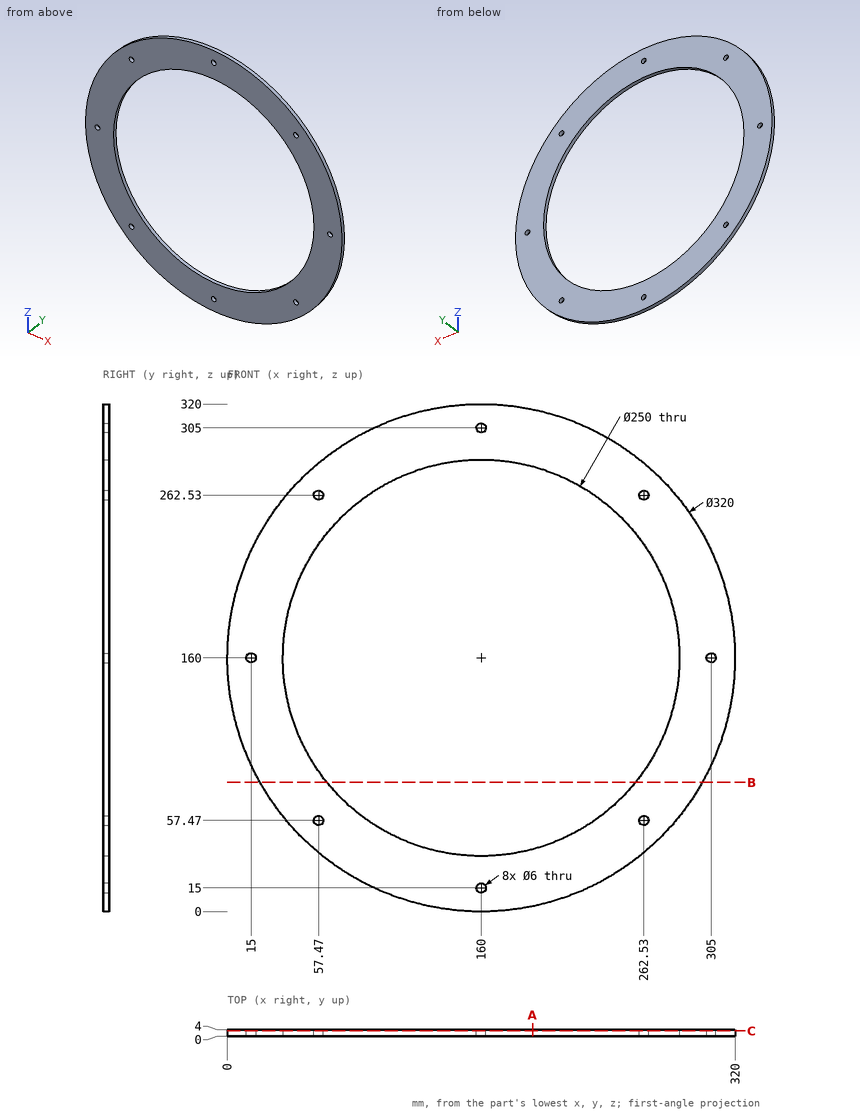
Answer from the drawing. Dimensions are ordinates in mm from the lowest x, y and z of the part. Coordinates: 2 decimals unless noted, no trailing zeros. Write each loop counter-clockwise with the first axis right and the second up, starting at its lowest first coordinate (ties: lowest second). Pieces come first, ordered by that corner, then holes. Notation, with made-up numbers: M -37,77 L -22,77 A6 cw -22,88 Z; hole C 19,-29 d7. An arc over 180 degrees is marked long. Put each result on its own line as item: value. Start each with the question number.
1. Flat-ended cylindrical pins translate along their axes: P1, Ø5.5, axis at x = 57.47, z = 262.53, coming from the -Y side; P2, Ø1, axis at x = 238.5, y = 3, coming from the -Z side; P3, Ø1.5, axis at y = 3, z = 108, coming from the -X side. Find the tip coordinate at first contact, or state that the pin passes through.
2. A cutting plane is placed at B-B on z = 81.5. Write down the section's boundary in (x, y).
3. A cutting plane is placed at A-A on x = 192.5. Write down the section's boundary in (y, z) (1 decimal).
4. A cutting plane is placed at C-C on y = 3.2. Count the separate pieces of the cut face and the enclosed holes in it, then the cut area to 3 significant figures.
5. Consider line 1 (X direction, y = 2.05, z = 55.5) (1 decimal); line 2 (X direction, y = 2.5, z = 179); line 3 (X direction, y = 3.15, z = 15) (1 decimal). Determine where each line is inside the solid, lowest interval first. Write a range as from..to.
Resolved:
1. P1: passes through
1. P2: stops at z = 20.3
1. P3: stops at x = 8.43
2. outline: M 20.58,0 L 62.72,0 L 62.72,4 L 20.58,4 Z; M 257.28,0 L 299.42,0 L 299.42,4 L 257.28,4 Z
3. outline: M 0,3.3 L 4,3.3 L 4,39.3 L 0,39.3 Z; M 0,280.7 L 4,280.7 L 4,316.7 L 0,316.7 Z
4. separate pieces: 1
4. enclosed holes: 9
4. area: 31,100 mm2
5. line 1: x = 38.8..55.2, 59.7..91.4, 228.6..260.3, 264.8..281.2
5. line 2: x = 1.13..36.45, 283.55..318.87
5. line 3: x = 92.4..157, 163..227.6
